Design review of the part built by this model. Coordinates are the model's own, in mm. Give positions to 0.01 mm unless a question says otherwise; leave off trailing zeros. Order: outer loops, then holes, each group sorted by start corner. A loop starts at its lowest first (then second) coordinate and runs counter-clockwise, first axis right, second up.
```python
from build123d import *

# Parameters (mm, degrees)
SKETCH1_R           = 10
SKETCH1_R_2         = 32.5
BOSS_EXTRUDE1_DEPTH = 0.5
SKETCH2_R           = 18
SKETCH2_R_2         = 3.5
CUT_EXTRUDE1_DEPTH  = 50
FILLET1_R           = 3


with BuildPart() as part:
    # Sketch1 → Boss-Extrude1 (new body)
    with BuildSketch(Plane(origin=(0, 0, 0), x_dir=(1, 0, 0), z_dir=(0, 1, 0))):
        with Locations((-21.213203436, -21.213203436)):
            Circle(SKETCH1_R)
        Circle(SKETCH1_R_2)
        with Locations((21.213203436, -21.213203436)):
            Circle(SKETCH1_R)
        with Locations((21.213203436, 21.213203436)):
            Circle(SKETCH1_R)
        with Locations((-21.213203436, 21.213203436)):
            Circle(SKETCH1_R)
    extrude(amount=BOSS_EXTRUDE1_DEPTH)

    # Sketch2 → Cut-Extrude1 (cut)
    with BuildSketch(Plane(origin=(0, 0.5, 0), x_dir=(1, 0, 0), z_dir=(0, 1, 0))):
        with Locations(Location((0, 0, 0), (0, 0, 270))):
            Circle(SKETCH2_R)
        with Locations(Location((21.213203436, 21.213203436, 0), (0, 0, 270))):
            Circle(SKETCH2_R_2)
        with Locations(Location((21.213203436, -21.213203436, 0), (0, 0, 270))):
            Circle(SKETCH2_R_2)
        with Locations(Location((-21.213203436, -21.213203436, 0), (0, 0, 270))):
            Circle(SKETCH2_R_2)
        with Locations(Location((-21.213203436, 21.213203436, 0), (0, 0, 270))):
            Circle(SKETCH2_R_2)
    extrude(amount=-CUT_EXTRUDE1_DEPTH, mode=Mode.SUBTRACT)

    # Fillet1
    fillet1_edges = [part.edges().sort_by_distance(p)[0] for p in [
        (-28.916041247, 0.25, -14.836190839),
        (-14.836190839, 0.25, -28.916041247),
        (14.836190839, 0.25, -28.916041247),
        (28.916041247, 0.25, -14.836190839),
        (28.916041247, 0.25, 14.836190839),
        (14.836190839, 0.25, 28.916041247),
        (-14.836190839, 0.25, 28.916041247),
        (-28.916041247, 0.25, 14.836190839),
    ]]
    fillet(fillet1_edges, radius=FILLET1_R)


solid = part.part
```
1. For line 1 along X through (y, z) = (0.35, 21.5); line 2 along X through (y, z) = (0.1, 0); line 3 along Z through (x, y) = (20, 0.2), list the stretches that pass through material, from the lowest coordinate up.
Recorded:
line 1: x = -31.21 to -24.7, -17.72 to 17.72, 24.7 to 31.21
line 2: x = -32.5 to -18, 18 to 32.5
line 3: z = -31.14 to -24.5, -17.93 to 17.93, 24.5 to 31.14
2. Take a section at C-C (y = 0.3). State how many separate pieces and enclosed holes the cut face has, then the cut area to 3 significant figures.
Recorded:
separate pieces: 1
enclosed holes: 5
area: 2,620 mm2
3. Take a section at A-A (x = 0). State the section outline as (y, z) points, then the cut area to 3 significant figures.
Recorded:
outline: (0, -32.5) - (0.5, -32.5) - (0.5, -18) - (0, -18) - close; (0, 18) - (0.5, 18) - (0.5, 32.5) - (0, 32.5) - close
area: 14.5 mm2
4. Draft analysis for pull direction Z (two halves, no side actions). For faces 1 (the face through (-15, 0.5, -15)), 2 (the face through (-24.318, 0.254, 22.828)), 3 (the face through (-0.2, 0.2, 32.5)), state which applies: pulls with the +Z half, pulls with the -Z half, needs draft (parallel to the pull), parting line crosses it, or undercut.
Recorded:
face 1: needs draft
face 2: undercut
face 3: pulls with the +Z half
5. Take a section at B-B (z = 0). State the section outline as (x, y) points.
Recorded:
outline: (-32.5, 0) - (-18, 0) - (-18, 0.5) - (-32.5, 0.5) - close; (18, 0) - (32.5, 0) - (32.5, 0.5) - (18, 0.5) - close
